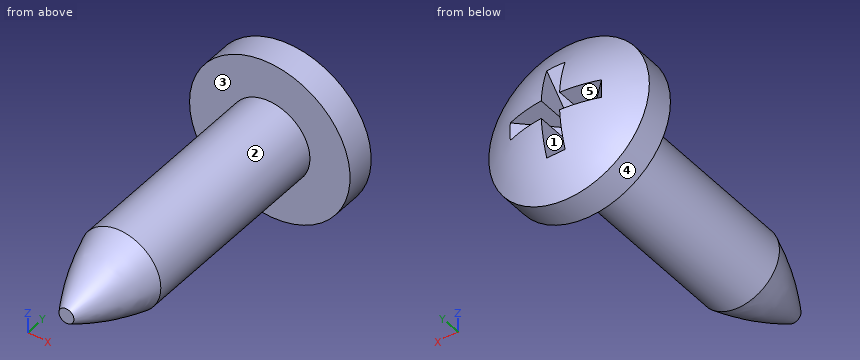
```python
from build123d import *

# Parameters (mm, degrees)
SKETCH2_R           = 1.75
BOSS_EXTRUDE1_DEPTH = 8.8
CUT_EXTRUDE1_DEPTH  = 0.4
CIRPATTERN1_COUNT   = 4


with BuildPart() as part:
    # Sketch1 → Revolve2 (revolve)
    with BuildSketch(Plane.XY, mode=Mode.PRIVATE) as revolve2_sk:
        with BuildLine():
            Line((0, 3.8596837944664038), (3.5000000000000013, 3.8596837944664038))
            Line((3.5000000000000013, 3.8596837944664038), (3.5000000000000013, 5.104743083003953))
            ThreePointArc((3.5000000000000013, 5.104743083003953), (1.8384255445316686, 5.9427548013385545), (8.7e-16, 6.231345910599472))
            Line((8.7e-16, 6.231345910599472), (0, 3.8596837944664038))
        make_face()
    revolve(revolve2_sk.sketch.rotate(Axis((0, 9.918972332015809, 0), (2.4e-16, -1, 0)), 180), axis=Axis((0, 9.918972332015809, 0), (2.4e-16, -1, 0)))

    # Sketch2 → Boss-Extrude1 (add)
    with BuildSketch(Plane.XZ.offset(-3.8596837944664033)):
        Circle(SKETCH2_R)
    extrude(amount=BOSS_EXTRUDE1_DEPTH)

    # Sketch3 → Revolve3 (revolve)
    with BuildSketch(Plane.XY, mode=Mode.PRIVATE) as revolve3_sk:
        with BuildLine():
            Line((-0.3268895580285352, -8.140316205533598), (0, -8.140316205533598))
            Line((0, -8.140316205533598), (-3.69e-15, -4.940316205533597))
            Line((-3.69e-15, -4.940316205533597), (-1.7500000000000084, -4.940316205533597))
            ThreePointArc((-1.7500000000000084, -4.940316205533597), (-1.148404721070234, -6.5892178123268526), (-0.3268895580285352, -8.140316205533598))
        make_face()
    revolve(revolve3_sk.sketch.rotate(Axis((0, 0, 0), (0, -1, 0)), 180), axis=Axis((0, 0, 0), (0, -1, 0)))

    # Sketch8 → Cut-Extrude1 (cut, symmetric)
    with BuildSketch(Plane.XY):
        with BuildLine():
            Line((-2, 5.888200160091848), (-0.3999999999999996, 4.331345910599471))
            Line((-0.3999999999999996, 4.331345910599471), (0.40000000000000047, 4.33134591059947))
            Line((0.40000000000000047, 4.33134591059947), (2, 5.8882001600918485))
            ThreePointArc((2, 5.8882001600918485), (3.4e-16, 6.231345910599467), (-2, 5.888200160091848))
        make_face()
    cut_extrude1 = extrude(amount=CUT_EXTRUDE1_DEPTH, both=True, mode=Mode.SUBTRACT)

    # CirPattern1: Cut-Extrude1 ×4 about axis
    cirpattern1_axis = Axis((3.1e-16, 0, 3.1e-16), (0, 1, 0))
    for i in range(1, CIRPATTERN1_COUNT):
        add(cut_extrude1.rotate(cirpattern1_axis, i * 360 / CIRPATTERN1_COUNT), mode=Mode.SUBTRACT)


solid = part.part
```
Read the model definition and answer for the solid it produces. Units are mm, in the model's axes. Face numbers are marked on the shaded views. A direction names the side the tool comes from. Round coordinates to 2 decimals unless told otherwise and drop trailing zeros. Write each loop counter-clockwise with the first axis right and the second up, starting at its lowest first coordinate (ties: lowest second). Pieces come first, ordered by that corner, then holes. Notation, with made-up numbers: (64, 34) -> (78, 34) arc R21 ccw to (78, 40) -> close; hole circle Ø6 at (-22.75, -2.5). An arc over 180 degrees is marked (long way). Answer in a Markdown table with one row per item. Add a question column.
1) Find section C-C, the plane z = 3. Determine the outline of the cut face in (x, y).
2) Which of the six approach directions +Z, -Z, +X, -X, +Y, -Y give full straight-line access (tool end or side, diameter ignored) to the marked faces 4 and 5?
3) Find section B-B, the plane y = -0.25. Determine the outline of the cut face in (x, z), and give its area (3 significant figures).
4) Find section D-D, the plane x = -3. Determine the outline of the cut face in (y, z), and give its area (3 significant figures).
5) Given P1, Ø4, axis at x = -2.5, y = -1, coming from the +Z side; P2, Ø1.5, axis at x = -0.5, z = -0.5, coming from the -Y side; P3, Ø1.3, axis at y = 5, z = 1, coming from the -X side; P4, Ø1.7, axis at y = 5, z = -1.5, coming from the -X side, each flat-ended and moving along its own axis, determine where each tip first touches the part or whether it passes through.
6) Consider line 1 (Z direction, x = 0, y = 4.75); line 2 (Z direction, x = 0, y = 2); line 3 (X direction, y = 1, z = 0.75). Determine where each line is inside the solid, lowest interval first.
7) Find section A-A, the plane y = 4.75. Determine the outline of the cut face in (x, z), and give its area (3 significant figures).
8) Determine the mould class of the marked faces 1, 2 and 3 for opening direction X: pulls with the +X half, pulls with the -X half, needs draft (parallel to the pull), parting line crosses it, or undercut.
Findings below:
| question | item | result |
|---|---|---|
| 1 | outline | (-1.8, 3.86) -> (1.8, 3.86) -> (1.8, 5.1) arc R5.2 ccw to (-1.8, 5.1) -> close |
| 2 | face 4 | +Y, -Y |
| 2 | face 5 | +Y |
| 3 | outline | circle Ø3.5 at (0, 0) |
| 3 | area | 9.62 mm² |
| 4 | outline | (3.86, -1.8) -> (5.1, -1.8) arc R5.2 ccw to (5.1, 1.8) -> (3.86, 1.8) -> close |
| 4 | area | 5.27 mm² |
| 5 | P1 | z = 1.68 |
| 5 | P2 | y = -8.14 |
| 5 | P3 | x = -3.48 |
| 5 | P4 | x = -3.44 |
| 6 | line 1 | -3.5 to -0.83, 0.83 to 3.5 |
| 6 | line 2 | -1.75 to 1.75 |
| 6 | line 3 | -1.58 to 1.58 |
| 7 | outline | circle Ø7 at (0, 0); hole (-0.83, -0.4) -> (-0.4, -0.4) -> (-0.4, -0.83) -> (0.4, -0.83) -> (0.4, -0.4) -> (0.83, -0.4) -> (0.83, 0.4) -> (0.4, 0.4) -> (0.4, 0.83) -> (-0.4, 0.83) -> (-0.4, 0.4) -> (-0.83, 0.4) -> close |
| 7 | area | 36.5 mm² |
| 8 | face 1 | undercut |
| 8 | face 2 | parting line crosses it |
| 8 | face 3 | needs draft |
